```python
from build123d import *

# Parameters (mm, degrees)
BOSS_EXTRUDE1_DEPTH = 22.5


with BuildPart() as part:
    # Sketch1 → Boss-Extrude1 (new, symmetric)
    with BuildSketch(Plane(origin=(0, 0, 0), x_dir=(0, 0, -1), z_dir=(1, 0, 0))):
        Polygon((0, 0), (1110, 0), (1110, 110), (200, 110), (0, 38), align=None)
    extrude(amount=BOSS_EXTRUDE1_DEPTH, both=True)


solid = part.part
```
Here's how the part is built. I have some questions about the finished solid (model axes, mm). Coordinates: 2 decimals unless noted, no trailing zeros. Loops run counter-clockwise (first coordinate to the right, second up) from the corner with the lowest first, then second, coordinate; pieces in that order, holes last. Notation, with made-up numbers: (65, -22) - (103, -22) arc R21 ccw to (103, -17) - close; hole circle Ø9 at (39, 85.25). An arc over 180 degrees is marked (long way). Return JSON: item names as keys, results as strings. Group by question number.
Item 1: If we section it at C-C on y = 76: Write out the boundary of the cut face in (x, z).
Item 2: If we section it at A-A on x = 14: Write out the boundary of the cut face in (y, z).
Item 3: I need wall thicknesses on line 1 (Y direction, x = -12.5, z = -107.5). Which ranges of the line are inside material? Lowest first, please. Write a range as from..to.
Item 4: If we section it at B-B on z = -106.5: Write out the boundary of the cut face in (x, y), and give its area (3 significant figures).
Calculated:
{
 "1": {"outline": "(-22.5, -1110) - (22.5, -1110) - (22.5, -105.56) - (-22.5, -105.56) - close"},
 "2": {"outline": "(0, -1110) - (110, -1110) - (110, -200) - (38, 0) - (0, 0) - close"},
 "3": {"line 1": "y = 0..76.7"},
 "4": {"outline": "(-22.5, 0) - (22.5, 0) - (22.5, 76.34) - (-22.5, 76.34) - close", "area": "3,440 mm^2"}
}
